```python
from build123d import *

# Parameters (mm, degrees)
BOSS_EXTRUDE1_DEPTH = 5


with BuildPart() as part:
    # Sketch1 → Boss-Extrude1 (new, symmetric)
    with BuildSketch(Plane.XY):
        with BuildLine():
            Line((0, 175), (0, 280))
            Line((0, 280), (80, 280))
            ThreePointArc((80, 280), (115.355339059, 265.355339059), (130, 230))
            Line((130, 230), (130, 0))
            Line((130, 0), (65, 0))
            Line((65, 0), (65, 150))
            Line((65, 150), (25, 150))
            Line((25, 150), (0, 175))
        make_face()
    extrude(amount=BOSS_EXTRUDE1_DEPTH, both=True)


solid = part.part
```
Input: part model. Units: mm. Frame: model coordinates. A direction names the side the tool comes from. Give positions to 0.01 mm unless a question says otherwise; leave off trailing zeros. Loops run counter-clockwise (first coordinate to the right, second up) from the corner with the lowest first, then second, coordinate; pieces in that order, holes last. Notation, with made-up numbers: M 72,-4.75 L 79,-4.75 A16 ccw 79,13.25 Z; hole C 65.5,78.5 d10. An arc over 180 degrees is marked long. Answer as CSV lines item,"result". Start each with the question number.
1. Pull-direction query (Y, two-part tool) for faces 1 (the face through (45, 150, 0)), 2 (the face through (0, 227, 0)), 3 (the face through (114.964, 265.742, 0.07)); classes: released by +Y, released by -Y, zero draft, split by the parting line, or undercut.
2. Section B-B on y = 111. Return loops of the section in (x, z), plus the area to 3 significant figures.
3. Line query: L1, parallel to X at y = 112, z = 1.75; L2, parallel to Y at x = 52.5, z = 3.5; L3, parallel to Y at x = 17, z = -2. Output: solid intervals per line, ascending.
4. Section C-C on x = 22. Return loops of the section in (y, z), plus the area to 3 significant figures.
5. Section A-A on z = -2. Return loops of the section in (x, y).
6. Reachability of faces 4 (the face through (39, 280, 0)), 5 (the face through (65, 74, 0)) from +Z, -Z, +X, -X, +Y, -Y: full face, straight path, thin tool, end or side. Return the list, or none.
7. Pin query (flat end, axial travel): P1, Ø5, axis at x = 39, z = 0.5, coming from the -Y side. Return the tip coordinate at first contact, or that it passes through.
Computed values:
1,face 1,"released by -Y"
1,face 2,"zero draft"
1,face 3,"released by +Y"
2,outline,"M 65,-5 L 130,-5 L 130,5 L 65,5 Z"
2,area,"650 mm²"
3,L1,"x = 65 to 130"
3,L2,"y = 150 to 280"
3,L3,"y = 158 to 280"
4,outline,"M 153,-5 L 280,-5 L 280,5 L 153,5 Z"
4,area,"1,270 mm²"
5,outline,"M 0,175 L 25,150 L 65,150 L 65,0 L 130,0 L 130,230 A50 ccw 80,280 L 0,280 Z"
6,face 4,"+Z, -Z, +X, -X, +Y"
6,face 5,"+Z, -Z, -X, -Y"
7,P1,"stops at y = 150"
